from build123d import *

# Parameters (mm, degrees)
SKETCH1_W           = 150
SKETCH1_H           = 350
BOSS_EXTRUDE1_DEPTH = 30
SKETCH2_R           = 25
SKETCH2_R_2         = 40
CUT_EXTRUDE1_DEPTH  = 30
FILLET1_R           = 2


with BuildPart() as part:
    # Sketch1 → Boss-Extrude1 (new body)
    with BuildSketch(Plane.XY):
        Rectangle(SKETCH1_W, SKETCH1_H)
    extrude(amount=BOSS_EXTRUDE1_DEPTH)

    # Sketch2 → Cut-Extrude1 (cut)
    with BuildSketch(Plane.XY.offset(30)):
        with Locations((0, 100)):
            Circle(SKETCH2_R)
        with Locations((0, -80)):
            Circle(SKETCH2_R_2)
    extrude(amount=-CUT_EXTRUDE1_DEPTH, mode=Mode.SUBTRACT)

    # Fillet1
    fillet1_edges = [part.edges().sort_by_distance(p)[0] for p in [
        (-75, 175, 15),
        (75, 175, 15),
        (75, -175, 15),
        (-75, -175, 15),
    ]]
    fillet(fillet1_edges, radius=FILLET1_R)


solid = part.part
Geometry: final body of the model. Coordinates: model frame, mm. Round coordinates to 2 decimals unless told otherwise and drop trailing zeros. Order: outer loops, then holes, each group sorted by start corner. A loop starts at its lowest first (then second) coordinate and runs counter-clockwise, first axis right, second up.
Q1. Material intervals for probe 1 along Y at (x, z) = (0, 17.5); probe 2 along Y at (x, z) = (31, 5.75); probe 3 along X at (y, z) = (-54.5, 13), sorted ascending.
Result sheet:
probe 1: y = -175 to -120, -40 to 75, 125 to 175
probe 2: y = -175 to -105.28, -54.72 to 175
probe 3: x = -75 to -30.82, 30.82 to 75
Q2. Section B-B, the plane y = 100. Output: boundary loops of the cut face in (x, z).
Result sheet:
outline: (-75, 0) - (-25, 0) - (-25, 30) - (-75, 30) - close; (25, 0) - (75, 0) - (75, 30) - (25, 30) - close
Q3. Section A-A, the plane x = 0. Output: boundary loops of the cut face in (y, z), and give its area (3 significant figures).
Result sheet:
outline: (-175, 0) - (-120, 0) - (-120, 30) - (-175, 30) - close; (-40, 0) - (75, 0) - (75, 30) - (-40, 30) - close; (125, 0) - (175, 0) - (175, 30) - (125, 30) - close
area: 6,600 mm2
Q4. Section D-D, the plane z = 14.5. Output: boundary loops of the cut face in (x, y), and give its area (3 significant figures).
Result sheet:
outline: (-75, -173) arc R2 ccw to (-73, -175) - (73, -175) arc R2 ccw to (75, -173) - (75, 173) arc R2 ccw to (73, 175) - (-73, 175) arc R2 ccw to (-75, 173) - close; hole circle Ø80 at (0, -80); hole circle Ø50 at (0, 100)
area: 45,500 mm2
Q5. Section C-C, the plane x = -32. Output: boundary loops of the cut face in (y, z).
Result sheet:
outline: (-175, 0) - (-104, 0) - (-104, 30) - (-175, 30) - close; (-56, 0) - (175, 0) - (175, 30) - (-56, 30) - close
Q6. Mould query, pull axis Y, two halves, no side actions, for faces 1 (the face through (-1, -175, 15)), 2 (the face through (-5.21, -40.34, 15.21)), 3 (the face through (-1, 175, 15)). Classes: released by +Y, released by -Y, zero draft, split by the parting line, or undercut.
Result sheet:
face 1: released by -Y
face 2: undercut
face 3: released by +Y
